The listing builds one solid part. Answer for the finished solid, in the listing's coordinates (mm). A direction names the side the tool comes from. Round coordinates to 2 decimals unless told otherwise and drop trailing zeros. Order: outer loops, then holes, each group sorted by start corner. A loop starts at its lowest first (then second) coordinate and runs counter-clockwise, first axis right, second up. Notation, with made-up numbers: (43, -26.75) -> (85, -26.75) arc R18 cw to (85, -1.75) -> close; hole circle Ø5 at (-18, 11). An arc over 180 degrees is marked (long way). Answer in a Markdown table with one row per item. Add a question column.
```python
from build123d import *

# Parameters (mm, degrees)
SKETCH_1_W             = 60
SKETCH_1_H             = 76
EXTRUDE_1_DEPTH        = 14
SKETCH_2_W             = 2
SKETCH_2_H             = 10
CUT_EXTRUDE_1_DEPTH    = 83.897527104
SKETCH_3_W             = 45
SKETCH_3_H             = 52
CUT_EXTRUDE_2_DEPTH    = 51.398412673
HOLE_WIZARD_M4_1_D     = 3.3
HOLE_WIZARD_M5_2_D     = 4.2
HOLE_WIZARD_M5_2_DEPTH = 12.4
HOLE_WIZARD_M5_2_TIP   = 1.2618073
SKETCH_8_W             = 5
SKETCH_8_H             = 5
CUT_EXTRUDE_3_DEPTH    = 51.398412673
FILLET_1_R             = 5
CHAMFER_1_SIZE         = 0.5


with BuildPart() as part:
    # 草图1 → 凸台-拉伸1 (new body)
    with BuildSketch(Plane.XY):
        Rectangle(SKETCH_1_W, SKETCH_1_H)
    extrude(amount=EXTRUDE_1_DEPTH)

    # 草图2 → 切除-拉伸1 (cut, through all)
    with BuildSketch(Plane(origin=(0, 38, 0), x_dir=(1, 0, 0), z_dir=(0, 1, 0))):
        with Locations((29, -7)):
            Rectangle(SKETCH_2_W, SKETCH_2_H)
    extrude(amount=-CUT_EXTRUDE_1_DEPTH, mode=Mode.SUBTRACT)

    # 草图3 → 切除-拉伸2 (cut, through all)
    with BuildSketch(Plane(origin=(0, 0, 0), x_dir=(-1, 0, 0), z_dir=(0, 0, -1))):
        with Locations((-7.5, 0)):
            Rectangle(SKETCH_3_W, SKETCH_3_H)
    extrude(amount=-CUT_EXTRUDE_2_DEPTH, mode=Mode.SUBTRACT)

    # M4 螺纹孔1 (through all)
    with Locations(Plane(origin=(0, 38, 0), x_dir=(1, 0, 0), z_dir=(0, 1, 0))):
        with Locations((23, -7)):
            Hole(HOLE_WIZARD_M4_1_D / 2)

    # M5 螺纹孔2
    with Locations(Plane.ZY.offset(30)):
        with Locations((7, 32.5), (7, -32.5)):
            Hole(HOLE_WIZARD_M5_2_D / 2, depth=HOLE_WIZARD_M5_2_DEPTH)
            with Locations((0, 0, -(HOLE_WIZARD_M5_2_DEPTH + HOLE_WIZARD_M5_2_TIP / 2))):  # 118° drill point
                Cone(0, HOLE_WIZARD_M5_2_D / 2, HOLE_WIZARD_M5_2_TIP, mode=Mode.SUBTRACT)

    # 草图8 → 切除-拉伸3 (cut, through all)
    with BuildSketch(Plane.XY.offset(14)):
        with Locations((-27.5, 0)):
            Rectangle(SKETCH_8_W, SKETCH_8_H)
    extrude(amount=-CUT_EXTRUDE_3_DEPTH, mode=Mode.SUBTRACT)

    # 圆角1
    fillet_1_edges = [part.edges().sort_by_distance(p)[0] for p in [
        (-15, -26, 7),
        (-15, 26, 7),
    ]]
    fillet(fillet_1_edges, radius=FILLET_1_R)

    # 倒角1
    chamfer_1_edges = [part.edges().sort_by_distance(p)[0] for p in [
        (-30, 20.25, 14),
        (30, -38, 1),
        (30, 38, 1),
        (0, -38, 14),
        (30, 32, 0),
        (30, 32, 14),
        (30, -26, 13),
        (30, -26, 1),
        (30, 26, 13),
        (30, 26, 1),
        (10, -26, 14),
        (10, -26, 0),
        (30, -32, 14),
        (0, -38, 0),
        (-30, 20.25, 0),
        (0, 38, 0),
        (30, -32, 0),
        (-30, -20.25, 0),
        (-30, -20.25, 14),
        (30, -38, 13),
        (-30, -38, 7),
        (-30, 38, 7),
        (30, 38, 13),
        (0, 38, 14),
        (10, 26, 14),
        (10, 26, 0),
        (-15, 0, 0),
        (-15, 0, 14),
        (-13.535533906, 24.535533906, 0),
        (-13.535533906, 24.535533906, 14),
        (-13.535533906, -24.535533906, 0),
        (-13.535533906, -24.535533906, 14),
    ]]
    chamfer(chamfer_1_edges, length=CHAMFER_1_SIZE)


solid = part.part
```
Item 1: The part is cut by section A-A, the plane x = 23. Give the vertices of the cut face in (y, z), and give its area (3 significant figures).
Item 2: The part is cut by section C-C, the plane z = 11. Give the vertices of the cut face in (x, y).
Item 3: Find the intervals of material crossed by probe 1 along Y at (x, z) = (-21.25, 7); probe 2 along Y at (x, z) = (14.5, 9.5); probe 3 along Z at (x, y) = (23, 31.5), in increasing order. Write a range as [from, to].
Item 4: A tool of negligible diameter and unlimited length cuts with its end or side. For faces 4 (the face through (29, 32, 2)), 5 (the face through (-13, 25, 7)), 6 (the face through (-13.591, -24.671, 0.365)), 7 (the face through (-13.676, -24.596, 13.642)), from which of +Z, -Z, +X, -X, +Y, -Y can it reach the whole face along a straight path? Write none if from no direction.
Item 5: The part is cut by section B-B, the plane x = 3.5. Give the vertices of the cut face in (y, z), and give its area (3 significant figures).
Item 6: For a pull along Z with two mould halves and no side action, classify faces 1 (the face through (-13.596, 24.676, 13.642)), 2 (the face through (-23.71, 30.45, 7.46)), 3 (the face through (10, 26, 7)) as released by +Z, released by -Z, zero draft, split by the parting line, or undercut.
Item 7: A flat-ended cylindrical pin translates along its axis: P1, Ø4.5, axis at x = 23, z = 7, coming from the -Y side. Find the tip coordinate at first contact, or state that the pin passes through.
Item 8: The part is cut by section D-D, the plane y = 15.5. Give the vertices of the cut face in (x, z).
Resolved:
| question | item | result |
|---|---|---|
| 1 | outline | (-38, 0.5) -> (-37.5, 0) -> (-26.5, 0) -> (-26, 0.5) -> (-26, 5.35) -> (-38, 5.35) -> close; (-38, 8.65) -> (-26, 8.65) -> (-26, 13.5) -> (-26.5, 14) -> (-37.5, 14) -> (-38, 13.5) -> close; (26, 0.5) -> (26.5, 0) -> (37.5, 0) -> (38, 0.5) -> (38, 5.35) -> (26, 5.35) -> close; (26, 8.65) -> (38, 8.65) -> (38, 13.5) -> (37.5, 14) -> (26.5, 14) -> (26, 13.5) -> close |
| 1 | area | 256 mm2 |
| 2 | outline | (-30, -37.5) -> (-29.5, -38) -> (28, -38) -> (28, -26) -> (-10, -26) arc R5 cw to (-15, -21) -> (-15, 21) arc R5 cw to (-10, 26) -> (28, 26) -> (28, 38) -> (-29.5, 38) -> (-30, 37.5) -> (-30, 2.5) -> (-25, 2.5) -> (-25, -2.5) -> (-30, -2.5) -> close |
| 3 | probe 1 | [-38, -34.6], [-30.4, 30.4], [34.6, 38] |
| 3 | probe 2 | [-38, -26], [26, 38] |
| 3 | probe 3 | [0, 5.35], [8.65, 14] |
| 4 | face 4 | +X, +Y, -Y |
| 4 | face 5 | +Z, -Z, +X |
| 4 | face 6 | -Z, +X |
| 4 | face 7 | +Z, +X |
| 5 | outline | (-38, 0.5) -> (-37.5, 0) -> (-26.5, 0) -> (-26, 0.5) -> (-26, 13.5) -> (-26.5, 14) -> (-37.5, 14) -> (-38, 13.5) -> close; (26, 0.5) -> (26.5, 0) -> (37.5, 0) -> (38, 0.5) -> (38, 13.5) -> (37.5, 14) -> (26.5, 14) -> (26, 13.5) -> close |
| 5 | area | 335 mm2 |
| 6 | face 1 | released by +Z |
| 6 | face 2 | undercut |
| 6 | face 3 | zero draft |
| 7 | P1 | y = -38 |
| 8 | outline | (-30, 0.5) -> (-29.5, 0) -> (-15.5, 0) -> (-15, 0.5) -> (-15, 13.5) -> (-15.5, 14) -> (-29.5, 14) -> (-30, 13.5) -> close |
